For this review, use the dimensioned drawing (mm, ordinates from the lowest corner) and the shaded views. Coordinates: 2 decimals unless noted, no trailing zeros. Loops run counter-clockwise (first coordinate to the right, second up) from the corner with the lowest first, then second, coordinate; pieces in that order, holes last. Notation, with made-up numbers: (-8.5, 52.25) -> (27.5, 52.25) arc R24 cw to (27.5, 67.25) -> close; hole circle Ø3 at (87, 79.5). An arc over 180 degrees is marked (long way). Use one line per item in the form item = value. Start each with the question number.
1. Wall thickness on line 1 (Y direction, x = 13, z = 4); line 2 (Y direction, x = 22, z = 4); line 3 (X direction, y = 14.5, z = 6.5): over which ranges is each line inside the solid? List them lowest first. Write a range as from..to.
2. The part is to be moulded in two halves that separate along Z. For the marked faces 1, 2 and 3, say which applies: released by +Z, released by -Z, zero draft, split by the parting line, or undercut.
3. Consider section A-A (z = 3). State the section outline as (x, y) points, then the cut area to 3 significant figures.
4. For pin 1 (4 mm diameter, centred on y = 18, z = 3, fed in from +X); pin 2 (2 mm diameter, centred on x = 23.5, z = 7.5, fed in from +Y) (3 decimals); pin 3 (6 mm diameter, centred on y = 19.5, z = 2.5, fed in from +X), all flat-tipped, find the tip position at first contact; note any pin that passes through.
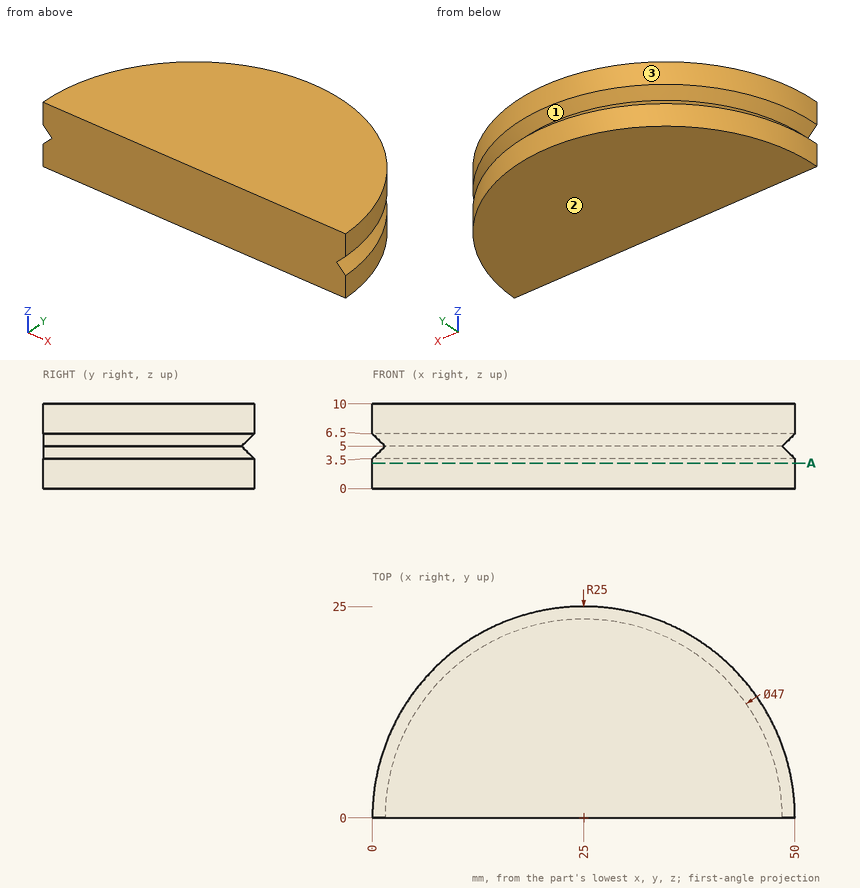
Geometry check:
q1.line_1 = 0..21.36
q1.line_2 = 0..24.32
q1.line_3 = 4.63..45.37
q2.face_1 = undercut
q2.face_2 = released by -Z
q2.face_3 = zero draft
q3.outline = (0, 0) -> (50, 0) arc R25 ccw to start
q3.area = 982 mm²
q4.pin_1 = 44.21
q4.pin_2 = 24.995
q4.pin_3 = 43.78
